```python
from build123d import *

# Parameters (mm, degrees)
SLIDE_PROFILE_SKETCH_W   = 120
SLIDE_PROFILE_SKETCH_H   = 55
SLIDE_PROFILE_SKETCH_R   = 15
SLIDE_PROFILE_SKETCH_R_2 = 5.5
SLIDE_BODY_35MM_DEPTH    = 35
FACE_RECESS_7MM_DEPTH    = 7
CURVED_POCKET_SKETCH_W   = 59
CURVED_POCKET_SKETCH_H   = 55
CURVED_POCKET_7MM_DEPTH  = 7
THROUGH_CUT_SKETCH_W     = 8
THROUGH_CUT_SKETCH_H     = 15
THROUGH_CUT_59MM_DEPTH   = 59


with BuildPart() as part:
    # Slide Profile Sketch → Slide Body 35mm (new body)
    with BuildSketch(Plane.XY):
        with Locations((0, 27.5)):
            Rectangle(SLIDE_PROFILE_SKETCH_W, SLIDE_PROFILE_SKETCH_H)
        with Locations((-15, 27.5)):
            Circle(SLIDE_PROFILE_SKETCH_R, mode=Mode.SUBTRACT)
        with Locations((28.282217915, 45)):
            Circle(SLIDE_PROFILE_SKETCH_R_2, mode=Mode.SUBTRACT)
        with Locations((28.282217915, 10)):
            Circle(SLIDE_PROFILE_SKETCH_R_2, mode=Mode.SUBTRACT)
    extrude(amount=SLIDE_BODY_35MM_DEPTH)

    # Face Recess Sketch → Face Recess 7mm (cut)
    with BuildSketch(Plane.XY.offset(35)):
        with BuildLine():
            Line((9.776428685, 55), (41.334840998, 55))
            ThreePointArc((41.334840998, 55), (45, 27.5), (41.334840998, 0))
            Line((41.334840998, 0), (9.776428685, 0))
            ThreePointArc((9.776428685, 0), (15, 27.5), (9.776428685, 55))
        make_face()
    extrude(amount=-FACE_RECESS_7MM_DEPTH, mode=Mode.SUBTRACT)

    # Curved Pocket Sketch → Curved Pocket 7mm (cut)
    with BuildSketch(Plane.XY.offset(35)):
        with Locations((-30.5, 27.5)):
            Rectangle(CURVED_POCKET_SKETCH_W, CURVED_POCKET_SKETCH_H)
    extrude(amount=-CURVED_POCKET_7MM_DEPTH, mode=Mode.SUBTRACT)

    # Through Cut Sketch → Through Cut 59mm (cut)
    with BuildSketch(Plane.ZY.offset(60)):
        with Locations((24, 27.5)):
            Rectangle(THROUGH_CUT_SKETCH_W, THROUGH_CUT_SKETCH_H)
    extrude(amount=-THROUGH_CUT_59MM_DEPTH, mode=Mode.SUBTRACT)


solid = part.part
```
The listing builds one solid part. Answer for the finished solid, in the listing's coordinates (mm). A direction names the side the tool comes from. Give positions to 0.01 mm unless a question says otherwise; leave off trailing zeros. Loops run counter-clockwise (first coordinate to the right, second up) from the corner with the lowest first, then second, coordinate; pieces in that order, holes last. Notation, with made-up numbers: M -35.75,-27.75 L 14.25,-27.75 A29 cw 14.25,1.25 Z; hole C 24.5,82 d4. An arc over 180 degrees is marked long. One line per item, written item: value.
1. Section D-D on z = 14 is taken. Determine the outline of the cut face in (x, y).
Found:
outline: M -60,0 L 60,0 L 60,55 L -60,55 Z; hole C -15,27.5 d30; hole C 28.28,10 d11; hole C 28.28,45 d11
2. Section B-B on z = 24 is taken. Determine the outline of the cut face in (x, y).
Found:
outline: M -60,0 L 60,0 L 60,55 L -60,55 L -60,35 L -27.99,35 A15 cw -2.01,35 L -1,35 L -1,32.89 A15 cw -1,22.11 L -1,20 L -2.01,20 A15 cw -27.99,20 L -60,20 Z; hole C 28.28,10 d11; hole C 28.28,45 d11
3. Find the intervals of material crossed by probe 1 along Y at (x, z) = (-15, 24.5); probe 2 along Y at (x, z) = (26, 7); probe 3 along X at (y, z) = (27.5, 11), in increasing order.
Found:
probe 1: 0 to 12.5, 42.5 to 55
probe 2: 0 to 5, 15 to 40, 50 to 55
probe 3: -60 to -30, 0 to 60
4. For a pull along Y with two mould halves and no side action, classify faces 4 (the face through (-1, 0, 13)), 5 (the face through (-31, 45, 28)), 6 (the face through (-44, 20, 24)) as pulls with the +Y half, pulls with the -Y half, needs draft (parallel to the pull), parting line crosses it, or undercut.
Found:
face 4: pulls with the -Y half
face 5: needs draft
face 6: undercut
5. Section A-A on y = 27.5 is taken. Determine the outline of the cut face in (x, z).
Found:
outline: M -60,0 L -30,0 L -30,20 L -60,20 Z; M 0,0 L 60,0 L 60,35 L 45,35 L 45,28 L 15,28 L 15,35 L 0,35 Z
6. For faces 1 (the face through (-31, 10, 28)), 2 (the face through (-44, 27, 20)), 3 (the face through (45, 28, 32)), determine the directions among +Z, -Z, +X, -X, +Y, -Y from which every point of the face is accessible in a straight line to the end or side of a thin tool.
Found:
face 1: +Z, -X, +Y, -Y
face 2: +Z, -X
face 3: +Z
7. Section C-C on x = -15 is taken. Determine the outline of the cut face in (y, z).
Found:
outline: M 0,0 L 12.5,0 L 12.5,28 L 0,28 Z; M 42.5,0 L 55,0 L 55,28 L 42.5,28 Z
8. Each of these flat-tipped pins is pushed along its axis until it touches: P1, Ø10.5, axis at x = 21.5, y = 16, coming from the +Z side; P2, Ø1.1, axis at x = -1.5, z = 24, coming from the -Y side; P3, Ø4.5, axis at y = 12, z = 30.5, coming from the -X side; P4, Ø6.5, axis at x = 28.28, y = 45, coming from the +Z side. Where does it stop, or does it pass through?
Found:
P1: z = 28
P2: y = 0
P3: x = -1
P4: through
